Could you check a few things on this model? Use its own coordinates, in mm. A direction names the side the tool comes from. Round coordinates to 2 decimals unless told otherwise and drop trailing zeros. Write each loop counter-clockwise with the first axis right and the second up, starting at its lowest first coordinate (ties: lowest second). Pieces come first, ordered by that corner, then holes. Notation, with made-up numbers: (-2.5, -21) -> (35.5, -21) arc R10 ccw to (35.5, -9) -> close; hole circle Ø2 at (-22, 87). An arc over 180 degrees is marked (long way). Return JSON: item names as keys, results as strings.
from build123d import *

# Parameters (mm, degrees)
SKETCH1_R           = 11.5
BOSS_EXTRUDE1_DEPTH = 30
SKETCH2_OUTSIDE_W   = 33.85
SKETCH2_OUTSIDE_H   = 33.85
CUT_EXTRUDE2_DEPTH  = 10
FILLET1_R           = 1
CUT_EXTRUDE3_DEPTH  = 35.124771062
SKETCH4_R           = 10.5
CUT_EXTRUDE4_DEPTH  = 18


with BuildPart() as part:
    # Sketch1 → Boss-Extrude1 (new body)
    with BuildSketch(Plane.XY):
        Circle(SKETCH1_R)
    extrude(amount=BOSS_EXTRUDE1_DEPTH)

    # Sketch2 outside → Cut-Extrude2 (cut)
    with BuildSketch(Plane.XY.offset(30)):
        Rectangle(SKETCH2_OUTSIDE_W, SKETCH2_OUTSIDE_H)
        Polygon((5.875781464, 9.885605302), (-5.623294591, 10.031378666), (-11.499076055, 0.145773364), (-5.875781464, -9.885605302), (5.623294591, -10.031378666), (11.499076055, -0.145773364), align=None, mode=Mode.SUBTRACT)
    extrude(amount=-CUT_EXTRUDE2_DEPTH, mode=Mode.SUBTRACT)

    # Fillet1
    fillet1_edges = [part.edges().sort_by_distance(p)[0] for p in [
        (8.68742876, 4.869915969, 30),
        (8.561185323, -5.088576015, 30),
        (-0.126243437, -9.958491984, 30),
        (-8.68742876, -4.869915969, 30),
        (-8.561185323, 5.088576015, 30),
        (0.126243437, 9.958491984, 30),
    ]]
    fillet(fillet1_edges, radius=FILLET1_R)

    # Sketch3 → Cut-Extrude3 (cut, through all)
    with BuildSketch(Plane.XY.offset(30)):
        with BuildLine():
            Line((0.5, 0), (0.5, 1.81976866))
            ThreePointArc((0.5, 1.81976866), (0.431071967, 2.991864898), (0.225238082, 4.147803077))
            Line((0.225238082, 4.147803077), (0, 5.088723004))
            Line((0, 5.088723004), (-0.225238082, 4.147803077))
            ThreePointArc((-0.225238082, 4.147803077), (-0.431071967, 2.991864898), (-0.5, 1.81976866))
            Line((-0.5, 1.81976866), (-0.5, 0))
            Line((-0.5, 0), (-0.5, -1.81976866))
            ThreePointArc((-0.5, -1.81976866), (-0.431071967, -2.991864898), (-0.225238082, -4.147803077))
            Line((-0.225238082, -4.147803077), (0, -5.088723004))
            Line((0, -5.088723004), (0.225238082, -4.147803077))
            ThreePointArc((0.225238082, -4.147803077), (0.431071967, -2.991864898), (0.5, -1.81976866))
            Line((0.5, -1.81976866), (0.5, 0))
        make_face()
    extrude(amount=-CUT_EXTRUDE3_DEPTH, mode=Mode.SUBTRACT)

    # Sketch4 → Cut-Extrude4 (cut)
    with BuildSketch(Plane(origin=(0, 0, 0), x_dir=(-1, 0, 0), z_dir=(0, 0, -1))):
        Circle(SKETCH4_R)
    extrude(amount=-CUT_EXTRUDE4_DEPTH, mode=Mode.SUBTRACT)


solid = part.part
1) Thinking about a two-plate mould opening in X: for faces 1 (the face through (-8.36, 4.87, 29.7)), 2 (the face through (8.4, 4.8, 29.7)), 3 (the face through (-0.43, 3.01, 24.08)), which applies, pulls with the +X half, pulls with the -X half, needs draft (parallel to the pull), parting line crosses it, or undercut?
Return value:
{"face 1": "pulls with the -X half", "face 2": "pulls with the +X half", "face 3": "undercut"}
2) I want a section at A-A, the plane z = 7.5. Please give me the cut outline in (x, y), and give its area (3 significant figures).
Return value:
{"outline": "circle Ø23 at (0, 0); hole circle Ø21 at (0, 0)", "area": "69.1 mm²"}
3) For faces 4 (the face through (-8.727, -4.8, 24.563)), 5 (the face through (0.042, 9.674, 29.699)), 6 (the face through (0.433, 2.976, 24.084)), 7 (the face through (-10, 3.2, 8.9)), which set-ups out of +Z, -Z, +X, -X, +Y, -Y let a thin tool reach every point of the face, with its end or its side?
Return value:
{"face 4": "+Z, -X, -Y", "face 5": "+Z, +X, +Y", "face 6": "+Z, -Z", "face 7": "-Z"}
4) Will these pins go through, and if not, where does the flat tip stop? pin 1 Ø3 at (x, z) = (5, 20) entering from -Y; pin 2 Ø4 at (y, z) = (0, 26) entering from +X; pin 3 Ø2 at (y, z) = (-3.5, 23) entering from +X.
Return value:
{"pin 1": "y = -10.95", "pin 2": "x = 11.5", "pin 3": "x = 10.1"}
5) If I drill on probe 1 along Y at (x, z) = (0, 9.5); probe 2 along Z at (x, y) = (4.25, 1.75); probe 3 along X at (y, z) = (-7.5, 6.5), over which ranges is the centre line in solid material (lowest first)? Write a range as [from, to].
Return value:
{"probe 1": "[-11.5, -10.5], [10.5, 11.5]", "probe 2": "[18, 30]", "probe 3": "[-8.72, -7.35], [7.35, 8.72]"}
